from build123d import *

# Parameters (mm, degrees)
BOSS_EXTRUDE1_DEPTH = 600
SKETCH4_OUTSIDE_W   = 1933.152
SKETCH4_OUTSIDE_H   = 942.352
SKETCH4_OUTSIDE_R   = 40
SKETCH4_OUTSIDE_R_2 = 50
CUT_EXTRUDE1_DEPTH  = 1121.500446229


with BuildPart() as part:
    # Sketch1 → Boss-Extrude1 (new body)
    with BuildSketch(Plane.XY):
        with BuildLine():
            Line((-1.216429586, 8), (-647.3, 8))
            Line((-647.3, 8), (-647.3, -8))
            Line((-647.3, -8), (-1.216429586, -8))
            ThreePointArc((-1.216429586, -8), (-0.542173275, -8.022756973), (0.12901423, -8.090924315))
            Line((0.12901423, -8.090924315), (417.518275664, -64.763596782))
            ThreePointArc((417.518275664, -64.763596782), (419.263363176, -64.940831871), (421.016429586, -65))
            Line((421.016429586, -65), (943.5, -65))
            Line((943.5, -65), (943.5, -49))
            Line((943.5, -49), (421.016429586, -49))
            ThreePointArc((421.016429586, -49), (420.342173275, -48.977243027), (419.67098577, -48.909075685))
            Line((419.67098577, -48.909075685), (2.281724336, 7.763596782))
            ThreePointArc((2.281724336, 7.763596782), (0.536636824, 7.940831871), (-1.216429586, 8))
        make_face()
    extrude(amount=BOSS_EXTRUDE1_DEPTH)

    # Sketch4 outside → Cut-Extrude1 (cut, through all)
    # profile 1 of 3: a face of its own
    with BuildSketch(Plane(origin=(0, 8, 0), x_dir=(1, 0, 0), z_dir=(0, 1, 0))):
        with Locations((148.1, -300)):
            Rectangle(SKETCH4_OUTSIDE_W, SKETCH4_OUTSIDE_H)
        with BuildLine():
            Line((849.441033389, -393.022786976), (-192.741176471, -487.726520609))
            ThreePointArc((-192.741176471, -487.726520609), (-228.733049722, -487.54676651), (-264.034655196, -480.529366519))
            ThreePointArc((-264.034655196, -480.529366519), (-446.549262984, -405.356942265), (-610.742483166, -295.798456192))
            ThreePointArc((-610.742483166, -295.798456192), (-641.798915546, -185.789833988), (-549.379294824, -118.521619672))
            Line((-549.379294824, -118.521619672), (-213.719470744, -111.540753082))
            ThreePointArc((-213.719470744, -111.540753082), (-203.220116273, -111.614875507), (-192.741176471, -112.273479391))
            Line((-192.741176471, -112.273479391), (849.441033389, -206.977213024))
            ThreePointArc((849.441033389, -206.977213024), (856.218024477, -210.53404245), (858.495022624, -217.84115701))
            Line((858.495022624, -217.84115701), (855.553845389, -250.207806915))
            ThreePointArc((855.553845389, -250.207806915), (801, -300), (855.553845389, -349.792193085))
            Line((855.553845389, -349.792193085), (858.495022624, -382.15884299))
            ThreePointArc((858.495022624, -382.15884299), (856.218024477, -389.46595755), (849.441033389, -393.022786976))
        make_face(mode=Mode.SUBTRACT)
    # profile 2 of 3: a face of its own
    with BuildSketch(Plane(origin=(0, 8, 0), x_dir=(1, 0, 0), z_dir=(0, 1, 0))):
        with Locations(Location((-547.3, -218.5, 0), (0, 0, 180))):
            Circle(SKETCH4_OUTSIDE_R)
    # profile 3 of 3: a face of its own
    with BuildSketch(Plane(origin=(0, 8, 0), x_dir=(1, 0, 0), z_dir=(0, 1, 0))):
        with Locations(Location((696, -300, 0), (0, 0, 180))):
            Circle(SKETCH4_OUTSIDE_R_2)
    extrude(amount=-CUT_EXTRUDE1_DEPTH, mode=Mode.SUBTRACT)


solid = part.part
Model file for the job. Use its own axes, mm. A direction names the side the tool comes from. Coordinates: 2 decimals unless noted, no trailing zeros. Loops run counter-clockwise (first coordinate to the right, second up) from the corner with the lowest first, then second, coordinate; pieces in that order, holes last. Notation, with made-up numbers: (33.25, 3.5) -> (49.25, 3.5) arc R11 cw to (49.25, 20.5) -> close; hole circle Ø9 at (28.25, 83.5). An arc over 180 degrees is marked (long way). Use one line per item in the form item = value. Start each with the question number.
(1) Cut at A-A on z = 322. Give the cut face in (x, y).
(2) Tool access for faces 5 (the flat face through (-257, -8, 297)), 6 (the flat face through (325.918, -36.441, 159.404)), 7 (the flat face through (594, -49, 298)): list every direction of +Z, -Z, +X, -X, +Y, -Y with a clear straight run to the whole face (end or side of a thin tool).
(3) Cut at B-B on x = 696. Give the cut face in (y, z), and give its area (3 significant figures).
(4) Probe probe 1 along Z at (x, y) = (851, -53); probe 2 along Y at (x, z) = (781.5, 208); probe 3 along Z at (x, y) = (-547.3, -1.5). List the from-to ranges inside material, lowest first. Write a range as from..to.
(5) Cut at D-D on x = 234.5. Give the cut face in (y, z), and give its area (3 significant figures).
(6) Cut at C-C on y = -25. Give the cut face in (x, z), and give its area (3 significant figures).
(7) Flat gauge pins, fed straight in: pin 1 (12 mm diameter, centred on x = -184.5, y = -3.5, fed in from +Z); pin 2 (10 mm diameter, centred on x = -351.5, y = -17, fed in from -Z); pin 3 (2 mm diameter, centred on y = -6.5, z = 314, fed in from -X). Where does each tip first touch, or does it go through?
(8) Pull direction Z, two halves, no side cores. Call faces 1 (the cylindrical face through (801.014, -56.888, 298.837)), 2 (the cylindrical face through (-584.25, 0.11, 203.18)), 3 (the cylindrical face through (-444.105, 0.112, 406.655)), 4 (the flat face through (213.9, -20.97, 297.62)): pulls with the +Z half, pulls with the -Z half, needs draft (parallel to the pull), parting line crosses it, or undercut.
Values:
q1.outline = (-577.4, -8) -> (-1.22, -8) arc R10 cw to (0.13, -8.09) -> (417.52, -64.76) arc R26 ccw to (421.02, -65) -> (651.1, -65) -> (651.1, -49) -> (421.02, -49) arc R10 cw to (419.67, -48.91) -> (2.28, 7.76) arc R26 ccw to (-1.22, 8) -> (-577.4, 8) -> close; (740.9, -65) -> (806.1, -65) -> (806.1, -49) -> (740.9, -49) -> close
q2.face_5 = +Z, -Z, -X, -Y
q2.face_6 = -Z, +X, +Y, -Y
q2.face_7 = +Z, -Z, +X, +Y
q3.outline = (-65, 193.03) -> (-49, 193.03) -> (-49, 250) -> (-65, 250) -> close; (-65, 350) -> (-49, 350) -> (-49, 406.97) -> (-65, 406.97) -> close
q3.area = 1,820 mm2
q4.probe_1 = 207.24..250, 350..392.76
q4.probe_2 = -65..-49
q4.probe_3 = 118.48..178.5, 258.5..343.78
q5.outline = (-39.91, 151.1) -> (-23.77, 151.1) -> (-23.77, 448.9) -> (-39.91, 448.9) -> close
q5.area = 4,810 mm2
q6.outline = (124.66, 141.12) -> (243.58, 151.92) -> (243.58, 448.08) -> (124.66, 458.88) -> close
q6.area = 36,500 mm2
q7.pin_1 = 487.52
q7.pin_2 = through
q7.pin_3 = -589.18
q8.face_1 = undercut
q8.face_2 = undercut
q8.face_3 = pulls with the +Z half
q8.face_4 = needs draft
